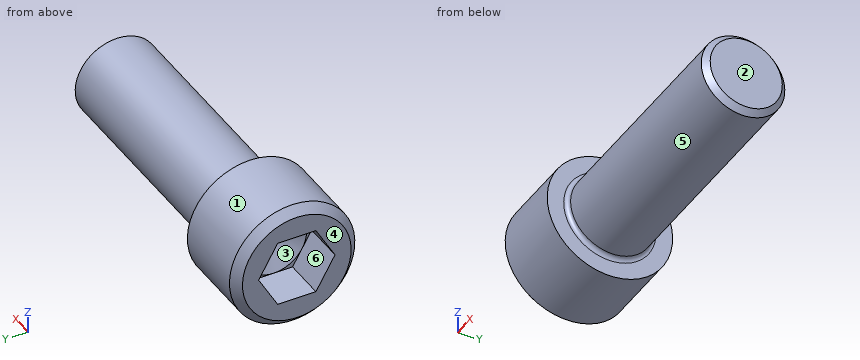
```python
from build123d import *

# Parameters (mm, degrees)
FILLET1_R   = 1.27
HEX_2_DEPTH = 12


with BuildPart() as part:
    # BodySke → Base-Revolve (revolve)
    with BuildSketch(Plane.XY, mode=Mode.PRIVATE) as base_revolve_sk:
        Polygon((0, 0), (0, 15.6), (2.4, 18), (24, 18), (24, 12), (92.352, 12), (94, 10.352), (94, 0), align=None)
    revolve(base_revolve_sk.sketch.rotate(Axis((-31.75, 0, 0), (1, 0, 0)), 90), axis=Axis((-31.75, 0, 0), (1, 0, 0)))

    # Fillet1
    fillet1_edges = [part.edges().sort_by_distance(p)[0] for p in [
        (24, 0, -12),
    ]]
    fillet(fillet1_edges, radius=FILLET1_R)

    # Sketch2 → Hex-PreBroach (revolve, cut)
    with BuildSketch(Plane.XY, mode=Mode.PRIVATE) as hex_prebroach_sk:
        Polygon((0, 9.5), (12, 9.5), (17.484827557, 0), (0, 0), align=None)
    revolve(hex_prebroach_sk.sketch.rotate(Axis((0, 0, 0), (1, 0, 0)), 90), axis=Axis((0, 0, 0), (1, 0, 0)), mode=Mode.SUBTRACT)

    # Sketch3 → Hex 2 (cut)
    with BuildSketch(Plane(origin=(0, 0, 0), x_dir=(0, 0.500000000000001, 0.866025403784438), z_dir=(-1, 0, 0))):
        Polygon((5.484827557, 9.5), (-5.484827557, 9.5), (-10.969655115, 0), (-5.484827557, -9.5), (5.484827557, -9.5), (10.969655115, 0), align=None)
    extrude(amount=-HEX_2_DEPTH, mode=Mode.SUBTRACT)


solid = part.part
```
Model file for the job. Use its own axes, mm. Face numbers are marked on the shaded views. A direction names the side the tool comes from. Coordinates: 2 decimals unless noted, no trailing zeros. Write each loop counter-clockwise with the first axis right and the second up, starting at its lowest first coordinate (ties: lowest second). Pieces come first, ordered by that corner, then holes. Notation, with made-up numbers: (31, 56.25) - (64, 56.25) arc R12 cw to (64, 72.25) - close; hole circle Ø6 at (65.25, 80). An arc over 180 degrees is marked (long way). Use a Markdown table: item, result. Add a question column.
Item 1: Drill centre lines: line 1 along X through (y, z) = (4.5, 14); line 2 along Z through (x, y) = (77, -0.5); line 3 along Z through (x, y) = (20.5, -9). Where is each one in solid material? Low to high.
Item 2: Drop flat-ended pins along their axis: pin 1 (10 mm diameter, centred on x = 36, z = -13.5, fed in from +Y); pin 2 (1.4 mm diameter, centred on y = 9.5, z = 2.5, fed in from -X); pin 3 (5 mm diameter, centred on x = 68.5, z = 2, fed in from -Y); pin 4 (3.5 mm diameter, centred on x = 5, y = 2.5, fed in from -Z). Give the stop position or say it passes through.
Item 3: Band-saw the part on A-A, the plane x = 32.5. Write the cut outline in (y, z), and give its area (3 significant figures).
Item 4: Two-plate mould, pull along Y, no slides. Class the marked faces 1, 2 and 3: pulls with the +Y half, pulls with the -Y half, needs draft (parallel to the pull), parting line crosses it, or undercut.
Item 5: Band-saw the part on B-B, the plane x = 15.5. Write the cut outline in (y, z), and give its area (3 significant figures).
Item 6: 3-axis set-ups, long thin cutter, end or side, ignore diameter. For the marked faces 4, 5 and 6: which of +Z, -Z, +X, -X, +Y, -Y reach the whole face in a straight line?
A:
| question | item | result |
|---|---|---|
| 1 | line 1 | x = 0 to 24 |
| 1 | line 2 | z = -11.99 to 11.99 |
| 1 | line 3 | z = -15.59 to 15.59 |
| 2 | pin 1 | stops at y = 8.47 |
| 2 | pin 2 | stops at x = 0 |
| 2 | pin 3 | stops at y = -12 |
| 2 | pin 4 | stops at z = -17.98 |
| 3 | outline | circle Ø24 at (0, 0) |
| 3 | area | 452 mm² |
| 4 | face 1 | parting line crosses it |
| 4 | face 2 | needs draft |
| 4 | face 3 | undercut |
| 5 | outline | circle Ø36 at (0, 0); hole circle Ø6.88 at (0, 0) |
| 5 | area | 981 mm² |
| 6 | face 4 | +Z, -Z, -X, +Y, -Y |
| 6 | face 5 | +X |
| 6 | face 6 | -X |
